```python
from build123d import *

# Parameters (mm, degrees)
BASE_PLATE_SKETCH_W       = 54
BASE_PLATE_SKETCH_H       = 84
BASE_PLATE_SKETCH_R       = 8
BASE_PLATE_DEPTH          = 20
BASE_PLATE_2_DEPTH        = 20
BEARING_BOSS_SKETCH_R     = 20
BEARING_BOSS_DEPTH        = 32
BORE_START                = -32
BORE_SKETCH_R             = 20
BORE_40_DEPTH             = 32
SIDE_CUT_DEPTH            = 32
CLEVIS_LUG_SKETCH_W       = 18
CLEVIS_LUG_SKETCH_H       = 48
CLEVIS_LUG_DEPTH          = 76
LUG_END_PROFILE_SKETCH_R  = 8
LUG_END_PROFILE_CUT_DEPTH = 76


with BuildPart() as part:
    # Base Plate Sketch → Base Plate (new body)
    with BuildSketch(Plane.XY):
        with Locations((-39, 19.918699187)):
            Rectangle(BASE_PLATE_SKETCH_W, BASE_PLATE_SKETCH_H)
        with Locations((-50, 19.918699187)):
            Circle(BASE_PLATE_SKETCH_R, mode=Mode.SUBTRACT)
        with Locations((-50, -8.081300813)):
            Circle(BASE_PLATE_SKETCH_R, mode=Mode.SUBTRACT)
    extrude(amount=-BASE_PLATE_DEPTH)



with BuildPart() as body_2:
    # Base Plate Sketch → Base Plate 2 (new body)
    with BuildSketch(Plane.XY):
        with Locations((39, 19.918699187)):
            Rectangle(BASE_PLATE_SKETCH_W, BASE_PLATE_SKETCH_H)
        with Locations(Location((50, -8.081300813, 0), (0, 0, 180))):
            Circle(BASE_PLATE_SKETCH_R, mode=Mode.SUBTRACT)
        with Locations(Location((50, 19.918699187, 0), (0, 0, 180))):
            Circle(BASE_PLATE_SKETCH_R, mode=Mode.SUBTRACT)
    extrude(amount=-BASE_PLATE_2_DEPTH)


with BuildPart() as part_1:
    add(part.part)

    add(body_2.part)  # Bearing Boss merges body 2
    # Bearing Boss Sketch → Bearing Boss (add)
    with BuildSketch(Plane(origin=(0, 0, -20), x_dir=(-1, 0, 0), z_dir=(0, 0, -1))):
        with BuildLine():
            Line((38, 61.918699187), (38, 25.918699187))
            Line((38, 25.918699187), (-38, 25.918699187))
            Line((-38, 25.918699187), (-38, 61.918699187))
            ThreePointArc((-38, 61.918699187), (0, 99.918699187), (38, 61.918699187))
        make_face()
        with Locations((0, 61.918699187)):
            Circle(BEARING_BOSS_SKETCH_R, mode=Mode.SUBTRACT)
    extrude(amount=-BEARING_BOSS_DEPTH)

    # Bore Sketch → Bore Ø40 (cut)
    with BuildSketch(Plane.XY.offset(12).offset(BORE_START)):
        with Locations(Location((0, 61.918699187, 0), (0, 0, 180))):
            Circle(BORE_SKETCH_R)
    extrude(amount=BORE_40_DEPTH, mode=Mode.SUBTRACT)

    # Side Cut Sketch → Side Cut (cut)
    with BuildSketch(Plane.XY):
        with BuildLine():
            ThreePointArc((-66, 33.918699187), (-46.201010127, 42.119709314), (-38, 61.918699187))
            Line((-38, 61.918699187), (-66, 61.918699187))
            Line((-66, 61.918699187), (-66, 33.918699187))
        make_face()
    side_cut = extrude(amount=-SIDE_CUT_DEPTH, mode=Mode.SUBTRACT)

    # Side Cut Mirror: Side Cut across plane
    add(side_cut.mirror(Plane(origin=(0, 0, 0), x_dir=(0, 0, 1), z_dir=(1, 0, 0))), mode=Mode.SUBTRACT)

    # Clevis Lug Sketch → Clevis Lug (add)
    with BuildSketch(Plane.XY):
        with Locations((-25, 1.918699187)):
            Rectangle(CLEVIS_LUG_SKETCH_W, CLEVIS_LUG_SKETCH_H)
    clevis_lug = extrude(amount=CLEVIS_LUG_DEPTH)

    # Clevis Lug Mirror: Clevis Lug across plane
    add(clevis_lug.mirror(Plane(origin=(0, 0, 0), x_dir=(0, 0, 1), z_dir=(1, 0, 0))))

    # Lug End Profile Sketch → Lug End Profile Cut (cut)
    with BuildSketch(Plane.ZY.offset(34)):
        with BuildLine():
            Line((76, 25.918699187), (12, 25.918699187))
            Line((12, 25.918699187), (64.834711668, 9.170766689))
            ThreePointArc((64.834711668, 9.170766689), (72.910371542, 3.3697471), (76, -6.081300813))
            Line((76, -6.081300813), (76, 25.918699187))
        make_face()
        with BuildLine():
            Line((76, -22.081300813), (76, -6.081300813))
            ThreePointArc((76, -6.081300813), (71.313708499, -17.395009312), (60, -22.081300813))
            Line((60, -22.081300813), (76, -22.081300813))
        make_face()
        with Locations((60, -6.081300813)):
            Circle(LUG_END_PROFILE_SKETCH_R)
    extrude(amount=-LUG_END_PROFILE_CUT_DEPTH, mode=Mode.SUBTRACT)


solid = part_1.part
```
Input: part model. Units: mm. Frame: model coordinates. A direction names the side the tool comes from. Give positions to 0.01 mm unless a question says otherwise; leave off trailing zeros. Order: outer loops, then holes, each group sorted by start corner. A loop starts at its lowest first (then second) coordinate and runs counter-clockwise, first axis right, second up. Notation, with made-up numbers: (79.25, 31.5) - (91.25, 31.5) arc R16 ccw to (91.25, 40.5) - close; hole circle Ø7 at (50, 36). An arc over 180 degrees is marked (long way). Put each result on its own line as item: value.
Item 1: Section query A-A, the plane x = 0. Return loops of the section in (y, z), then the cut area to 3 significant figures.
Found:
outline: (25.92, -20) - (41.92, -20) - (41.92, 12) - (25.92, 12) - close; (81.92, -20) - (99.92, -20) - (99.92, 12) - (81.92, 12) - close
area: 1,090 mm^2
Item 2: Access query for faces 1 (the flat face through (-1, 39, 12)), 2 (the flat face through (-14, 2, 0)), 3 (the flat face through (-38, 44, 6)), 4 (the flat face through (36, 25.919, 6)). Directions: +Z, -Z, +X, -X, +Y, -Y. A direction counts if a zero-diameter tool reaches every point of the face in a straight line with its end or side. Return the directions, or none.
Found:
face 1: +Z, +X, -X, +Y
face 2: +Z, -Y
face 3: +Z, -X, +Y, -Y
face 4: +Z, +X, -Y
Item 3: Draft query along Z for faces 5 (the cylindrical face through (-25, -6, 52)), 6 (the flat face through (-12, 2, -10)), 7 (the flat face through (-25.13, 17.66, 38.05)). Return one class per face: +Z half, -Z half, draft (parallel to the pull), parting line (faces both ways), or undercut.
Found:
face 5: undercut
face 6: draft
face 7: +Z half
Item 4: Ray query, L1, parallel to Y at x = 0, z = -1; L2, parallel to X at y = 17, z = 7.5; L3, parallel to Y at x = -50, z = -9. Return the intervals inside material, ascending. Write a range as from..to.
Found:
L1: y = 25.92..41.92, 81.92..99.92
L2: x = -34..-16, 16..34
L3: y = -22.08..-16.08, -0.08..11.92, 27.92..38.94
Item 5: Section query D-D, the plane x = -30.5. Return loops of the section in (y, z), then the cut area to 3 significant figures.
Found:
outline: (-22.08, -20) - (84.58, -20) - (84.58, 12) - (25.92, 12) - (9.17, 64.83) arc R16 ccw to (-22.08, 60) - close; hole circle Ø16 at (-6.08, 60)
area: 5,550 mm^2
Item 6: Section query C-C, the plane z = 63. Return loops of the section in (x, y).
Found:
outline: (-34, -21.8) - (-16, -21.8) - (-16, -13.5) - (-34, -13.5) - close; (-34, 1.33) - (-16, 1.33) - (-16, 9.75) - (-34, 9.75) - close; (16, -21.8) - (34, -21.8) - (34, -13.5) - (16, -13.5) - close; (16, 1.33) - (34, 1.33) - (34, 9.75) - (16, 9.75) - close
Item 7: Section query B-B, the plane y = 52.5. Return loops of the section in (x, z), then the cut area to 3 significant figures.
Found:
outline: (-39.63, -20) - (-17.64, -20) - (-17.64, 12) - (-38, 12) - (-38, 0) - (-39.63, 0) - close; (17.64, -20) - (39.63, -20) - (39.63, 0) - (38, 0) - (38, 12) - (17.64, 12) - close
area: 1,370 mm^2
Item 8: Contact query for flat-ended pins moving along their axis: pin 1 (3.5 mm diameter, centred on y = 36.5, z = 6, fed in from +X); pin 2 (13 mm diameter, centred on y = 43.5, z = 4.5, fed in from -X); pin 3 (3 mm diameter, centred on x = -1.5, z = 3.5, fed in from +Y). Output: stop coordinate, or through.
Found:
pin 1: stops at x = 38
pin 2: stops at x = -50.19
pin 3: stops at y = 99.92
